Build history of the part. All positions in model axes, mm. Give positions to 0.01 mm unless a question says otherwise; leave off trailing zeros. Order: outer loops, then holes, each group sorted by start corner. A loop starts at its lowest first (then second) coordinate and runs counter-clockwise, first axis right, second up. Notation, with made-up numbers: M -26.75,-12 L -11.75,-12 A22 ccw -11.75,17 Z; hole C 50.5,-18 d3. An arc over 180 degrees is marked long. One line per item, written item: value.
from build123d import *

# Parameters (mm, degrees)
BASEKEY_DEPTH = 4.5
CHAMFER1_SIZE = 0.6


with BuildPart() as part:
    # Sketch1 → BaseKey (new, symmetric)
    with BuildSketch(Plane.XY):
        with BuildLine():
            Line((-56, 7), (0, 7))
            ThreePointArc((0, 7), (7, 0), (0, -7))
            Line((0, -7), (-56, -7))
            ThreePointArc((-56, -7), (-63, 0), (-56, 7))
        make_face()
    extrude(amount=BASEKEY_DEPTH, both=True)

    # Chamfer1
    chamfer1_edges = [part.edges().sort_by_distance(p)[0] for p in [
        (7, 0, 4.5),
        (-28, 7, 4.5),
        (-63, 0, 4.5),
        (-28, 7, -4.5),
        (7, 0, -4.5),
        (-28, -7, -4.5),
        (-63, 0, -4.5),
        (-28, -7, 4.5),
    ]]
    chamfer(chamfer1_edges, length=CHAMFER1_SIZE)


solid = part.part
1) Drill centre lines: probe 1 along X at (y, z) = (5.5, 3.75); probe 2 along X at (y, z) = (2.5, 3.5); probe 3 along Y at (x, z) = (-23, 4). Where is each one in solid material? Low to high. Write a range as from..to.
Check values:
probe 1: -60.33..4.33
probe 2: -62.54..6.54
probe 3: -6.9..6.9
2) Pin check, flat tip, straight feed: pin 1 (1 mm diameter, centred on y = 3.5, z = -0.5, fed in from -X). Stop position of the tip, or through.
Check values:
pin 1: x = -62.32
3) Saw through at A-A, the plane z = -1.5. Write the cut outline in (x, y).
Check values:
outline: M -56,-7 L 0,-7 A7 ccw 0,7 L -56,7 A7 ccw Z
